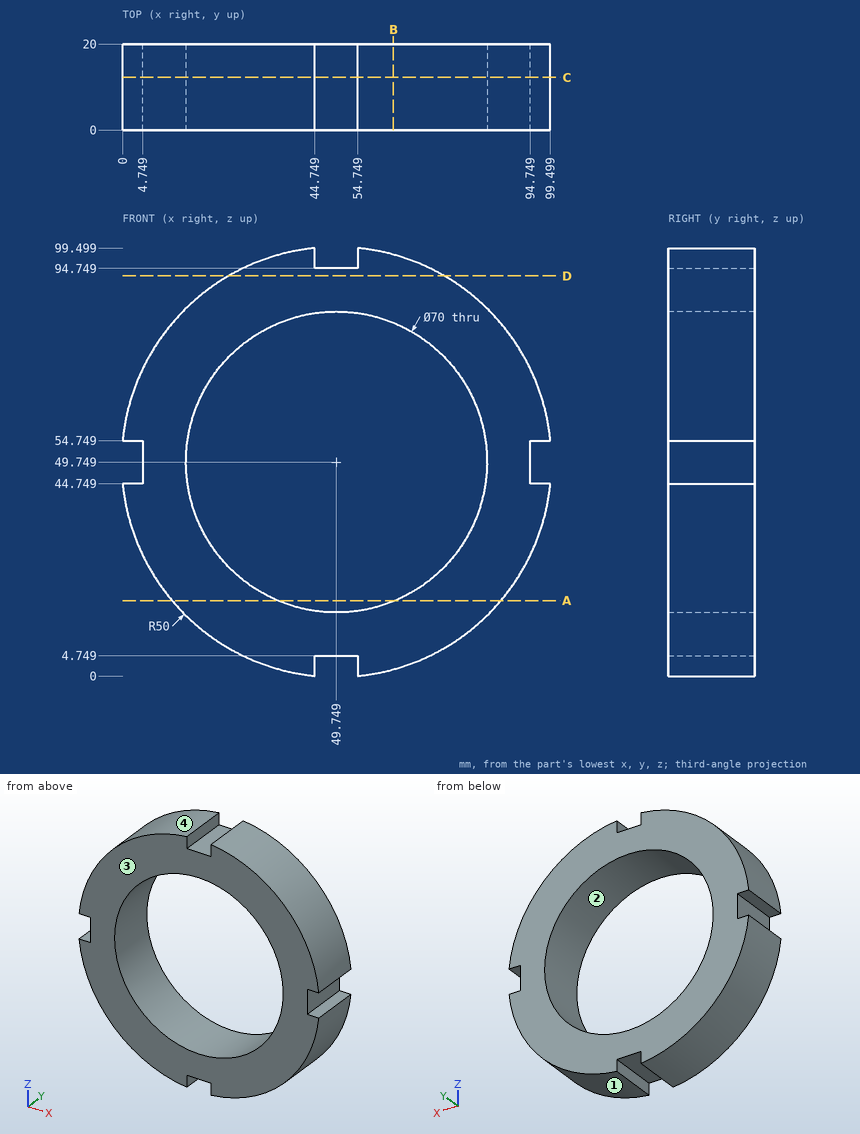
Geometry check sheet. Reference: drawing and pictorial views, mm from the part's lowest x, y, z. Round coordinates to 2 decimals unless told otherwise and drop trailing zeros. Write each loop counter-clockwise with the first axis right and the second up, starting at its lowest first coordinate (ties: lowest second). Pieces come first, ordered by that corner, then holes. Notation, with made-up numbers: (61, 89.25) -> (82, 89.25) arc R27 ccw to (82, 123.25) -> close; hole circle Ø4 at (79.5, -4). An arc over 180 degrees is marked (long way). Answer as CSV lines item,"result". Start each with the question number.
1) Section check A-A on z = 17.5. Enter the section's corners in (x, y).
2) Material ranges on line 1 (Z direction, x = 48.5, y = 17.25); line 2 (X direction, y = 14.75, z = 34) (1 decimal); line 3 (X direction, y = 13.25, z = 80.5) (1 decimal), recorded low to high. Write a range as from..to.
3) Go/stop test with flat-tipped pins: P1, Ø5, axis at x = 48.5, y = 12.5, coming from the +Z side; P2, Ø2, axis at x = 12, y = 5.5, coming from the -Z side (1 decimal); P3, Ø3, axis at x = 48.5, y = 12.5, coming from the -Z side. Record where each tip stops, or that it passes through.
4) Section check C-C on y = 12.25. Enter the section's corners in (x, z).
5) Section check B-B on x = 63. Enter the section's corners in (y, z) (1 decimal).
6) Section check D-D on z = 93. Enter the section's corners in (x, y), and give its area (3 significant figures).
7) Release check for a two-part mould opening along Z. For the marked faces 1, 2, 3 and 4 record: pulls with the +Z half, pulls with the -Z half, needs draft (parallel to the pull), parting line crosses it, or undercut.
Found:
1,outline,"(11.54, 0) -> (36.15, 0) -> (36.15, 20) -> (11.54, 20) -> close; (63.35, 0) -> (87.96, 0) -> (87.96, 20) -> (63.35, 20) -> close"
2,line 1,"z = 4.75..14.77, 84.73..94.75"
2,line 2,"x = 2.3..18.5, 81..97.2"
2,line 3,"x = 10.3..33, 66.5..89.2"
3,P1,"stops at z = 94.75"
3,P2,"stops at z = 15.8"
3,P3,"stops at z = 4.75"
4,outline,"(0, 44.75) arc R50 ccw to (44.75, 0) -> (44.75, 4.75) -> (54.75, 4.75) -> (54.75, 0) arc R50 ccw to (99.5, 44.75) -> (94.75, 44.75) -> (94.75, 54.75) -> (99.5, 54.75) arc R50 ccw to (54.75, 99.5) -> (54.75, 94.75) -> (44.75, 94.75) -> (44.75, 99.5) arc R50 ccw to (0, 54.75) -> (4.75, 54.75) -> (4.75, 44.75) -> close; hole circle Ø70 at (49.75, 49.75)"
5,outline,"(0, 1.5) -> (20, 1.5) -> (20, 17.4) -> (0, 17.4) -> close; (0, 82.1) -> (20, 82.1) -> (20, 98) -> (0, 98) -> close"
6,outline,"(24.66, 0) -> (74.84, 0) -> (74.84, 20) -> (24.66, 20) -> close"
6,area,"1,000 mm^2"
7,face 1,"pulls with the -Z half"
7,face 2,"undercut"
7,face 3,"needs draft"
7,face 4,"pulls with the +Z half"
